```python
from build123d import *

# Parameters (mm, degrees)
SKETCH1_R                  = 215
BOSS_EXTRUDE1_DEPTH        = 40
F_16_0_16_DIAMETER_HOLE1_D = 16
SKETCH7_R                  = 110
SKETCH7_R_2                = 40
BOSS_EXTRUDE2_DEPTH        = 85


with BuildPart() as part:
    # Sketch1 → Boss-Extrude1 (new body)
    with BuildSketch(Plane(origin=(0, 0, 0), x_dir=(1, 0, 0), z_dir=(0, 1, 0))):
        with Locations(Location((0, 0, 0), (0, 0, 270))):
            Circle(SKETCH1_R)
    extrude(amount=BOSS_EXTRUDE1_DEPTH)

    # Ø16.0 (16) Diameter Hole1 (through all)
    with Locations(Plane(origin=(0, 40, 0), x_dir=(1, 0, 0), z_dir=(0, 1, 0))):
        with Locations((200, 0), (190.211303259, -61.803398875), (161.803398875, -117.557050458), (117.557050458, -161.803398875), (61.803398875, -190.211303259), (0, -200), (-61.803398875, -190.211303259), (-117.557050458, -161.803398875), (-161.803398875, -117.557050458), (-190.211303259, -61.803398875), (-200, 0), (-190.211303259, 61.803398875), (-161.803398875, 117.557050458), (-117.557050458, 161.803398875), (-61.803398875, 190.211303259), (0, 200), (61.803398875, 190.211303259), (117.557050458, 161.803398875), (161.803398875, 117.557050458), (190.211303259, 61.803398875)):
            Hole(F_16_0_16_DIAMETER_HOLE1_D / 2)

    # Sketch7 → Boss-Extrude2 (add)
    with BuildSketch(Plane.XZ):
        with Locations(Location((0, 0, 0), (0, 0, 90))):
            Circle(SKETCH7_R)
        with Locations(Location((0, 0, 0), (0, 0, 270))):
            Circle(SKETCH7_R_2, mode=Mode.SUBTRACT)
    extrude(amount=BOSS_EXTRUDE2_DEPTH)


solid = part.part
```
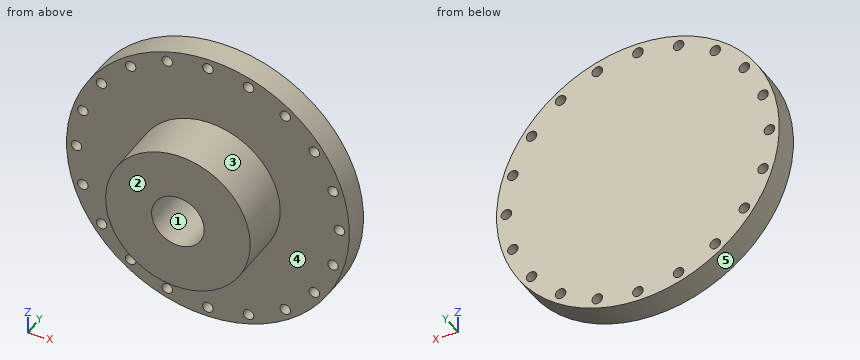
Could you check a few things on this model? Use its own coordinates, in mm. Face numbers are marked on the shaded views. A direction names the side the tool comes from. Coordinates: 2 decimals unless noted, no trailing zeros. Order: outer loops, then holes, each group sorted by start corner. A loop starts at its lowest first (then second) coordinate and runs counter-clockwise, first axis right, second up. Notation, with made-up numbers: M 8,48.5 L 17,48.5 A16 ccw 17,64.5 Z; hole C -18,77.25 d9. An arc over 180 degrees is marked long. Use one line per item in the form item = value. Start each with the question number.
1. Suppose I cut it at B-B on z = 0. Write out the boundary of the cut face in (x, y).
2. For pin 1 (18.5 mm diameter, centred on x = -200, z = 0, fed in from -Y); pin 2 (14.5 mm diameter, centred on x = -61.8, z = 190.21, fed in from +Y); pin 3 (6 mm diameter, centred on y = -19, z = -71.5, fed in from -X); pin 4 (2 mm diameter, centred on x = 80.5, y = -53, fed in from -Z), each with a flat end and sliding along its axis, tell me the tip position at first contact or that it passes through.
3. Suppose I cut it at C-C on y = -20.5. Write out the boundary of the cut face in (x, z), then the cut area to 3 significant figures.
4. Suppose I cut it at D-D on x = 96. Write out the boundary of the cut face in (y, z), then the cut area to 3 significant figures.
5. Suppose I cut it at A-A on x = 0. Write out the boundary of the cut face in (y, z), then the cut area to 3 significant figures.
6. Please list where these lines run through material, in increasing order: line 1 (X direction, y = 13.5, z = 64.5); line 2 (Z direction, x = -110.5, y = 23); line 3 (Y direction, x = -53, z = 157).
7. On a 3-axis mill with a long thin cutter (end or side, diameter ignored), from which of +Z, -Z, +X, -X, +Y, -Y can I reach the whole of each face in a straight line? I mean the marked faces 4 and 5. Say none if no direction works.
8. We'd pull the mould along X, two halves only. Please class the marked faces 1, 2 and 3: +X half, -X half, draft (parallel to the pull), parting line (faces both ways), or undercut.
Geometry says:
q1.outline = M -215,0 L -208,0 L -208,40 L -215,40 Z; M -192,0 L -110,0 L -110,-85 L -40,-85 L -40,0 L 40,0 L 40,-85 L 110,-85 L 110,0 L 192,0 L 192,40 L -192,40 Z; M 208,0 L 215,0 L 215,40 L 208,40 Z
q2.pin_1 = 0
q2.pin_2 = through
q2.pin_3 = -86.07
q2.pin_4 = -76.02
q3.outline = C 0,0 d220; hole C 0,0 d80
q3.area = 33,000 mm^2
q4.outline = M -85,-53.7 L 0,-53.7 L 0,-192.38 L 40,-192.38 L 40,192.38 L 0,192.38 L 0,53.7 L -85,53.7 Z
q4.area = 24,500 mm^2
q5.outline = M -85,-110 L 0,-110 L 0,-192 L 40,-192 L 40,192 L 0,192 L 0,110 L -85,110 L -85,40 L 0,40 L 0,-40 L -85,-40 Z; M 0,-215 L 40,-215 L 40,-208 L 0,-208 Z; M 0,208 L 40,208 L 40,215 L 0,215 Z
q5.area = 27,800 mm^2
q6.line_1 = -205.1 to -197.74, -182.68 to 182.68, 197.74 to 205.1
q6.line_2 = -184.43 to -165.57, -158.04 to 158.04, 165.57 to 184.43
q6.line_3 = 0 to 40
q7.face_4 = -Y
q7.face_5 = +Y, -Y
q8.face_1 = undercut
q8.face_2 = draft
q8.face_3 = parting line
